Part model, mm, in its own coordinate system. A direction names the side the tool comes from. Coordinates: 2 decimals unless noted, no trailing zeros. Loops run counter-clockwise (first coordinate to the right, second up) from the corner with the lowest first, then second, coordinate; pieces in that order, holes last. Notation, with made-up numbers: M 48.5,-29 L 66.5,-29 A14 ccw 66.5,-8 Z; hole C -8,54.25 d9. An arc over 180 degrees is marked long. Answer as CSV lines item,"result". Start each with the question number.
from build123d import *

# Parameters (mm, degrees)
SKETCH_1_W             = 122
SKETCH_1_H             = 122
EXTRUDE_1_DEPTH        = 15.5
SKETCH_2_W             = 148.5
SKETCH_2_H             = 148.5
EXTRUDE_2_DEPTH        = 13.5
SKETCH_3_W             = 100
SKETCH_3_H             = 5
CUT_EXTRUDE_1_DEPTH    = 109.936334618
PATTERN_LINEAR_1_COUNT = 11
PATTERN_LINEAR_1_PITCH = 10
MM_1_D                 = 5
MM_1_DEPTH             = 10
MM_1_TIP               = 1.502151548
HOLE_WIZARD_M4_1_D     = 3.3
HOLE_WIZARD_M4_1_DEPTH = 10.1
HOLE_WIZARD_M4_1_TIP   = 0.991420021


with BuildPart() as part:
    # 草图1 → 凸台-拉伸1 (new body)
    with BuildSketch(Plane.XY):
        Rectangle(SKETCH_1_W, SKETCH_1_H)
    extrude(amount=EXTRUDE_1_DEPTH)

    # 草图2 → 凸台-拉伸2 (add)
    with BuildSketch(Plane.XY.offset(15.5)):
        Rectangle(SKETCH_2_W, SKETCH_2_H)
    extrude(amount=EXTRUDE_2_DEPTH)

    # 草图3 → 切除-拉伸1 (cut, through all)
    with BuildSketch(Plane.XY.offset(29)):
        with Locations((0, 54.25)):
            Rectangle(SKETCH_3_W, SKETCH_3_H)
    cut_extrude_1 = extrude(amount=-CUT_EXTRUDE_1_DEPTH, mode=Mode.SUBTRACT)

    # 阵列(线性)1: 切除-拉伸1 ×11
    with Locations(*[(0, -i * PATTERN_LINEAR_1_PITCH, 0) for i in range(1, PATTERN_LINEAR_1_COUNT)]):
        add(cut_extrude_1, mode=Mode.SUBTRACT)

    # 大小mm 暗销孔1
    with Locations(Plane(origin=(0, 0, 15.5), x_dir=(-1, 0, 0), z_dir=(0, 0, -1))):
        with Locations((-65.5, 65.5), (0, 65.5), (65.5, 65.5), (65.5, 0), (-65.5, 0), (-65.5, -65.5), (0, -65.5), (65.5, -65.5)):
            Hole(MM_1_D / 2, depth=MM_1_DEPTH)
            with Locations((0, 0, -(MM_1_DEPTH + MM_1_TIP / 2))):  # 118° drill point
                Cone(0, MM_1_D / 2, MM_1_TIP, mode=Mode.SUBTRACT)

    # M4 螺纹孔1
    with Locations(Plane(origin=(0, 0, 0), x_dir=(-1, 0, 0), z_dir=(0, 0, -1))):
        with Locations((-52.5, 52.5), (52.5, 52.5), (52.5, -52.5), (-52.5, -52.5)):
            Hole(HOLE_WIZARD_M4_1_D / 2, depth=HOLE_WIZARD_M4_1_DEPTH)
            with Locations((0, 0, -(HOLE_WIZARD_M4_1_DEPTH + HOLE_WIZARD_M4_1_TIP / 2))):  # 118° drill point
                Cone(0, HOLE_WIZARD_M4_1_D / 2, HOLE_WIZARD_M4_1_TIP, mode=Mode.SUBTRACT)


solid = part.part
Q1. Tool access for faces 3 (the face through (-61, -1, 8)), 4 (the face through (-53.716, -51.385, 5.121)), 5 (the face through (-1, 21.75, 15)): list every direction of +Z, -Z, +X, -X, +Y, -Y with a clear straight run to the whole face (end or side of a thin tool).
Q2. Two-plate mould, pull along Y, no slides. Class faces 1 (the face through (-50, 44, 15)), 2 (the face through (-1, 1, 29)): +Y half, -Y half, draft (parallel to the pull), parting line (faces both ways), or undercut.
Q3. Slice it at D-D, the plane x = 5. State how many separate pieces and enclosed holes the cut face has, and give its area (3 significant figures).
Q4. Wall check: L1, parallel to Y at x = 65.5, z = 22.75; L2, parallel to Y at x = 52.5, z = 3. Give the ranges that are in metal, low to high.
Q5. Slice it at A-A, the plane y = 14. Write the cut outline in (x, z), and give its area (3 significant figures).
Q6. Flat gauge pins, fed straight in: P1, Ø5.5, axis at y = -46.5, z = 7.5, coming from the -X side; P2, Ø12, axis at x = -21.5, z = 3.5, coming from the +Y side. Where does each tip first touch, or does it go through?
Q7. Slice it at B-B, the plane y = -20. Write the cut outline in (x, z).
Solved:
1,face 3,"-Z, -X, +Y, -Y"
1,face 4,"-Z"
1,face 5,"+Z, -Z"
2,face 1,"undercut"
2,face 2,"draft"
3,separate pieces,"12"
3,enclosed holes,"0"
3,area,"2,300 mm2"
4,L1,"y = -74.25 to -68, -63 to -2.5, 2.5 to 63, 68 to 74.25"
4,L2,"y = -61 to -54.15, -50.85 to 50.85, 54.15 to 61"
5,outline,"M -74.25,15.5 L -61,15.5 L -61,0 L -50,0 L -50,29 L -74.25,29 Z; M 50,0 L 61,0 L 61,15.5 L 74.25,15.5 L 74.25,29 L 50,29 Z"
5,area,"996 mm2"
6,P1,"stops at x = -61"
6,P2,"stops at y = 61"
7,outline,"M -74.25,15.5 L -61,15.5 L -61,0 L 61,0 L 61,15.5 L 74.25,15.5 L 74.25,29 L -74.25,29 Z"
